Verification items for the finished model (mm, model axes). A direction names the side the tool comes from. Give positions to 0.01 mm unless a question says otherwise; leave off trailing zeros. Order: outer loops, then holes, each group sorted by start corner. A loop starts at its lowest first (then second) coordinate and runs counter-clockwise, first axis right, second up.
from build123d import *

# Parameters (mm, degrees)
EXTRUDE_1_DEPTH     = 1300
SKETCH_2_R          = 2.75
CUT_EXTRUDE_1_DEPTH = 10


with BuildPart() as part:
    # 草图1 → 拉伸-薄壁1 (new body)
    with BuildSketch(Plane.XY):
        Polygon((54, 6), (54, 0), (0, 0), (0, -15), (-1.5, -15), (-1.5, 1.5), (52.5, 1.5), (52.5, 6), align=None)
    extrude(amount=EXTRUDE_1_DEPTH)

    # 草图2 → 切除-拉伸1 (cut)
    with BuildSketch(Plane(origin=(0, 0, 0), x_dir=(0, 0, -1), z_dir=(1, 0, 0))):
        with Locations(Location((-1250, -7.5, 0), (0, 0, 90))):
            Circle(SKETCH_2_R)
        with Locations(Location((-950, -7.5, 0), (0, 0, 90))):
            Circle(SKETCH_2_R)
        with Locations(Location((-650, -7.5, 0), (0, 0, 90))):
            Circle(SKETCH_2_R)
        with Locations(Location((-350, -7.5, 0), (0, 0, 90))):
            Circle(SKETCH_2_R)
        with Locations(Location((-50, -7.5, 0), (0, 0, 90))):
            Circle(SKETCH_2_R)
    extrude(amount=-CUT_EXTRUDE_1_DEPTH, mode=Mode.SUBTRACT)


solid = part.part
(1) Section check B-B, the plane x = 14. Enter the section's corners in (y, z), then the cut area to 3 significant figures.
Solved:
outline: (0, 0) - (1.5, 0) - (1.5, 1300) - (0, 1300) - close
area: 1,950 mm2
(2) Section check A-A, the plane z = 511. Enter the section's corners in (x, y).
Solved:
outline: (-1.5, -15) - (0, -15) - (0, 0) - (54, 0) - (54, 6) - (52.5, 6) - (52.5, 1.5) - (-1.5, 1.5) - close
(3) Set-up check for faces 1 (the flat face through (27, 0, 641)), 2 (the flat face through (25, 1.5, 641)), 3 (the flat face through (22.3, 0.2, 1300)): record each of +Z, -Z, +X, -X, +Y, -Y from which the full face is reachable in a straight line by a thin tool's end or side.
Solved:
face 1: +Z, -Z, +X, -Y
face 2: +Z, -Z, -X, +Y
face 3: +Z, +X, -X, +Y, -Y
(4) Scan lines: line 1 (Z direction, x = -0.45, y = -7.5); line 2 (Y direction, x = -1.1, z = 1250); line 3 (X direction, y = -10, z = 702). Record each from-to range of solid material in increasing order.
Solved:
line 1: z = 0 to 47.25, 52.75 to 347.25, 352.75 to 647.25, 652.75 to 947.25, 952.75 to 1247.25, 1252.75 to 1300
line 2: y = -15 to -10.25, -4.75 to 1.5
line 3: x = -1.5 to 0
(5) Go/stop test with flat-tipped pins: pin 1 (3 mm diameter, centred on y = -5, z = 660.5, fed in from +X); pin 2 (2 mm diameter, centred on x = 4.5, z = 941.5, fed in from -Y); pin 3 (1 mm diameter, centred on x = 31.5, y = 0, fed in from -Z); pin 4 (16 mm diameter, centred on x = 28.5, z = 835.5, fed in from +Y). Record where each tip stops, or that it passes through.
Solved:
pin 1: stops at x = 0
pin 2: stops at y = 0
pin 3: stops at z = 0
pin 4: stops at y = 1.5
